Can you work these out from the model? Positions are in its coordinate system, mm. Coordinates: 2 decimals unless noted, no trailing zeros. Order: outer loops, then holes, each group sorted by start corner. A loop starts at its lowest first (then second) coordinate and runs counter-clockwise, first axis right, second up. Notation, with made-up numbers: (64, 16) - (95, 16) arc R26 ccw to (95, 38) - close; hole circle Ø5 at (26.5, 23.5). An arc over 180 degrees is marked (long way). Use a Markdown table: item, result. Add a question column.
(1) For pin 1 Ø3 at (x, z) = (134, 5) entering from +Y; pin 2 Ø1.5 at (x, z) = (104, 5) entering from -Y; pin 3 Ø7 at (x, y) = (190, -275) entering from +Z, each with a flat end and sliding along its axis, tell me the tip position at first contact or that it passes through.
(2) We'd pull the mould along Y, two halves only. Please class faces 1 (the flat face through (112.83, -61.5, 2.96)), 2 (the flat face through (67.6, -105.25, 2.96)), 3 (the flat face through (128, -134, 0)), 4 (the cylindrical face through (186.868, -272.128, 2.958)): pulls with the +Y half, pulls with the -Y half, needs draft (parallel to the pull), parting line crosses it, or undercut.
(3) I want a section at B-B (z = 2.95). List the corners of the cut face in (x, y) for me, and give its area (3 significant figures).
(4) I want a section at A-A (y = -275). List the corners of the cut face in (x, z) for me.
(5) I want a section at C-C (x = 97). List the corners of the cut face in (y, z) for me.
(6) If I drill on L1, parallel to X at y = -275, z = 1.8; L2, parallel to X at y = -210, z = 4.45; L3, parallel to Y at x = 189, z = 4.7, over which ranges is the centre line in solid material (lowest first)? Write a range as [from, to].
(7) I want a section at D-D (y = -44). List the corners of the cut face in (x, z) for me.
```python
from build123d import *

# Parameters (mm, degrees)
SKETCH_1_R      = 3
SKETCH_1_R_2    = 4.25
EXTRUDE_1_DEPTH = 6
CHAMFER_1_SIZE  = 5


with BuildPart() as part:
    # 草图1 → 凸台-拉伸1 (new body)
    with BuildSketch(Plane.XY):
        with BuildLine():
            Line((16.006925776, 19.203601933), (212.409696086, -144.505507303))
            ThreePointArc((212.409696086, -144.505507303), (221.696524755, -156.547022178), (225, -171.390550009))
            Line((225, -171.390550009), (225, -295))
            Line((225, -295), (155, -295))
            Line((155, -295), (155, -201.097000919))
            ThreePointArc((155, -201.097000919), (153.895948255, -195.4487603), (150.746317055, -190.631979669))
            Line((150.746317055, -190.631979669), (-17.910528426, -17.441702082))
            ThreePointArc((-17.910528426, -17.441702082), (-18.347356822, 16.981592907), (16.006925776, 19.203601933))
        make_face()
        Circle(SKETCH_1_R, mode=Mode.SUBTRACT)
        with Locations((190, -275)):
            Circle(SKETCH_1_R_2, mode=Mode.SUBTRACT)
        with Locations((190, -225)):
            Circle(SKETCH_1_R_2, mode=Mode.SUBTRACT)
        with Locations((190, -175)):
            Circle(SKETCH_1_R_2, mode=Mode.SUBTRACT)
    extrude(amount=EXTRUDE_1_DEPTH)

    # 倒角1
    chamfer_1_edges = [part.edges().sort_by_distance(p)[0] for p in [
        (225, -295, 3),
        (155, -295, 3),
    ]]
    chamfer(chamfer_1_edges, length=CHAMFER_1_SIZE)


solid = part.part
```
Answers follow:
| question | item | result |
|---|---|---|
| 1 | pin 1 | stops at y = -77.9 |
| 1 | pin 2 | stops at y = -143.4 |
| 1 | pin 3 | passes through |
| 2 | face 1 | pulls with the +Y half |
| 2 | face 2 | pulls with the -Y half |
| 2 | face 3 | needs draft |
| 2 | face 4 | undercut |
| 3 | outline | (-17.91, -17.44) - (150.75, -190.63) arc R15 cw to (155, -201.1) - (155, -290) - (160, -295) - (220, -295) - (225, -290) - (225, -171.39) arc R35 ccw to (212.41, -144.51) - (16.01, 19.2) arc R25 ccw to start; hole circle Ø6 at (0, 0); hole circle Ø8.5 at (190, -275); hole circle Ø8.5 at (190, -225); hole circle Ø8.5 at (190, -175) |
| 3 | area | 25,500 mm² |
| 4 | outline | (155, 0) - (185.75, 0) - (185.75, 6) - (155, 6) - close; (194.25, 0) - (225, 0) - (225, 6) - (194.25, 6) - close |
| 5 | outline | (-135.44, 0) - (-48.31, 0) - (-48.31, 6) - (-135.44, 6) - close |
| 6 | L1 | x = [155, 185.75], [194.25, 225] |
| 6 | L2 | x = [155, 225] |
| 6 | L3 | y = [-295, -279.13], [-270.87, -229.13], [-220.87, -179.13], [-170.87, -124.99] |
| 7 | outline | (7.95, 0) - (91.83, 0) - (91.83, 6) - (7.95, 6) - close |
